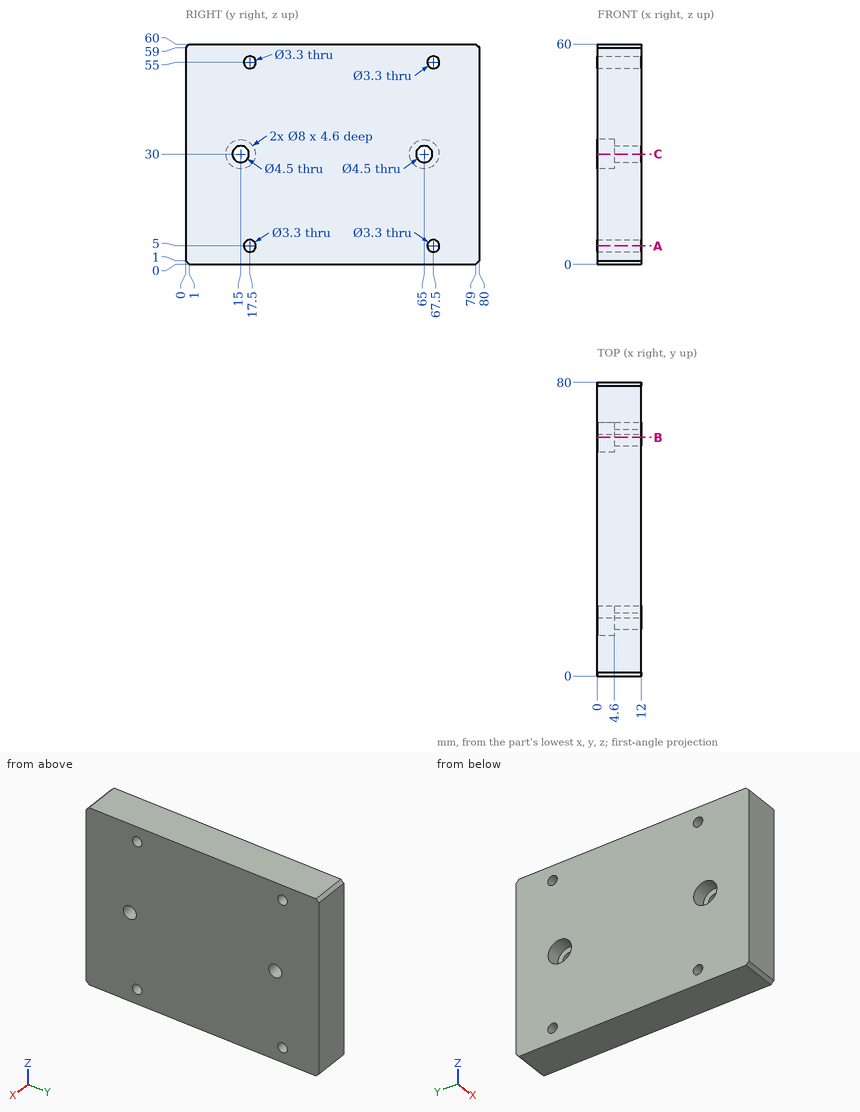
Source: three-view drawing plus pictorial views. Frame: mm from the lowest corner of the part. Coordinates: 2 decimals unless noted, no trailing zeros. Order: outer loops, then holes, each group sorted by start corner. A loop starts at its lowest first (then second) coordinate and runs counter-clockwise, first axis right, second up. Notation, with made-up numbers: M 11,-1.5 L 48,-1.5 A15 ccw 48,26.5 Z; hole C 73.25,77 d7. An arc over 180 degrees is marked long. Write each question's results on one line, items separated by ' | '. Start each with the question number.
1. Material intervals for L1, parallel to Y at x = 3.05, z = 30; L2, parallel to Y at x = 8.5, z = 30; L3, parallel to Z at x = 8.5, y = 65, sorted ascending.
2. Section A-A, the plane z = 5. Return the cut outline in (x, y), then the cut area to 3 significant figures.
3. Section C-C, the plane z = 30. Return the cut outline in (x, y), then the cut area to 3 significant figures.
4. Pin query (flat end, axial travel): pin 1 (4 mm diameter, centred on y = 16, z = 30.5, fed in from -X). Return the tip coordinate at first contact, or that it passes through.
5. Section B-B, the plane y = 65. Return the cut outline in (x, z).
Solution:
1) L1: 0 to 11, 19 to 61, 69 to 80 | L2: 0 to 12.75, 17.25 to 62.75, 67.25 to 80 | L3: 0 to 27.75, 32.25 to 60
2) outline: M 0,0 L 12,0 L 12,15.85 L 0,15.85 Z; M 0,19.15 L 12,19.15 L 12,65.85 L 0,65.85 Z; M 0,69.15 L 12,69.15 L 12,80 L 0,80 Z | area: 881 mm²
3) outline: M 0,0 L 12,0 L 12,12.75 L 4.6,12.75 L 4.6,11 L 0,11 Z; M 0,19 L 4.6,19 L 4.6,17.25 L 12,17.25 L 12,62.75 L 4.6,62.75 L 4.6,61 L 0,61 Z; M 0,69 L 4.6,69 L 4.6,67.25 L 12,67.25 L 12,80 L 0,80 Z | area: 820 mm²
4) pin 1: x = 4.6
5) outline: M 0,0 L 12,0 L 12,27.75 L 4.6,27.75 L 4.6,26 L 0,26 Z; M 0,34 L 4.6,34 L 4.6,32.25 L 12,32.25 L 12,60 L 0,60 Z
